from build123d import *

# Parameters (mm, degrees)
SKETCH1_R           = 273.05
SKETCH1_R_2         = 117.475
BOSS_EXTRUDE1_DEPTH = 127
FILLET1_R           = 5


with BuildPart() as part:
    # Sketch1 → Boss-Extrude1 (new body)
    with BuildSketch(Plane.XY):
        Circle(SKETCH1_R)
        Circle(SKETCH1_R_2, mode=Mode.SUBTRACT)
    extrude(amount=BOSS_EXTRUDE1_DEPTH)

    # Fillet1
    fillet1_edges = [part.edges().sort_by_distance(p)[0] for p in [
        (-273.05, 0, 0),
        (-273.05, 0, 127),
        (-117.475, 0, 0),
        (-117.475, 0, 127),
    ]]
    fillet(fillet1_edges, radius=FILLET1_R)


solid = part.part
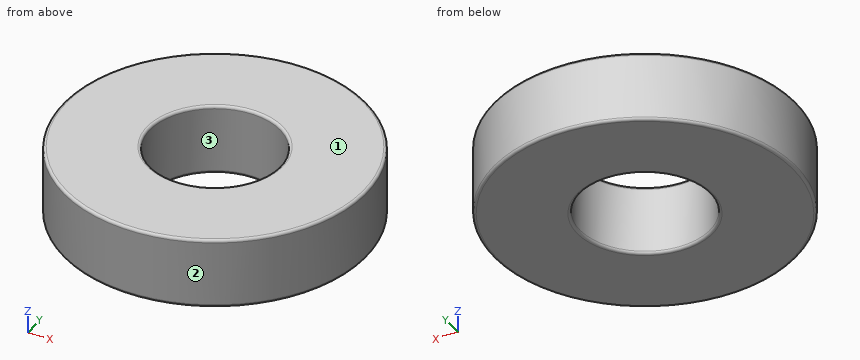
Design review of the part built by this model. Coordinates are the model's own, in mm. Face numbers are marked on the shaded views. Coordinates: 2 decimals unless noted, no trailing zeros. Loops run counter-clockwise (first coordinate to the right, second up) from the corner with the lowest first, then second, coordinate; pieces in that order, holes last. Notation, with made-up numbers: M 32,35 L 47,35 A18 ccw 47,55 Z; hole C 6,13 d3. An arc over 180 degrees is marked long. Use one line per item in the form item = value.
(1) Clearance check with flat-ended pins moving along their axes: P1, Ø2, axis at x = 66.5, y = -137.5, coming from the -Z side; P2, Ø6, axis at x = 216, z = 35, coming from the +Y side; P3, Ø1.5, axis at y = 65, z = 59, coming from the -X side; P4, Ø1, axis at y = -178, z = 56.5, coming from the -X side. State where each tip first meets the part, or that it passes through.
Return value:
P1 = 0
P2 = 170.84
P3 = -265.38
P4 = -207.49
(2) For line 1 along Y through (x, z) = (0, 33) (3 decimals); line 2 along Y through (x, z) = (-21, 69); line 3 along X through (y, z) = (56, 6.5), list the stretches that pass through material, from the lowest coordinate up. Write a range as from..to.
Return value:
line_1 = -273.05..-117.475, 117.475..273.05
line_2 = -272.24..-115.58, 115.58..272.24
line_3 = -267.25..-103.27, 103.27..267.25
(3) Consider section A-A (y = 0). Write out the cut boundary in (x, z) (3 decimals).
Return value:
outline = M -273.05,5 A5 ccw -268.05,0 L -122.475,0 A5 ccw -117.475,5 L -117.475,122 A5 ccw -122.475,127 L -268.05,127 A5 ccw -273.05,122 Z; M 117.475,5 A5 ccw 122.475,0 L 268.05,0 A5 ccw 273.05,5 L 273.05,122 A5 ccw 268.05,127 L 122.475,127 A5 ccw 117.475,122 Z
(4) Consider section C-C (z = 32). Write out the cut boundary in (x, y) (3 decimals).
Return value:
outline = C 0,0 d546.1; hole C 0,0 d234.95
(5) Draft analysis for pull direction X (two halves, no side actions). For the marked faces 1, 2 and 3, state which applies: pulls with the +X half, pulls with the -X half, needs draft (parallel to the pull), parting line crosses it, or undercut.
Return value:
face_1 = needs draft
face_2 = parting line crosses it
face_3 = undercut
